For this review, use the dimensioned drawing (mm, ordinates from the lowest corner) and the shaded views. Give positions to 0.01 mm unless a question says otherwise; leave off trailing zeros. Order: outer loops, then holes, each group sorted by start corner. A loop starts at its lowest first (then second) coordinate and runs counter-clockwise, first axis right, second up.
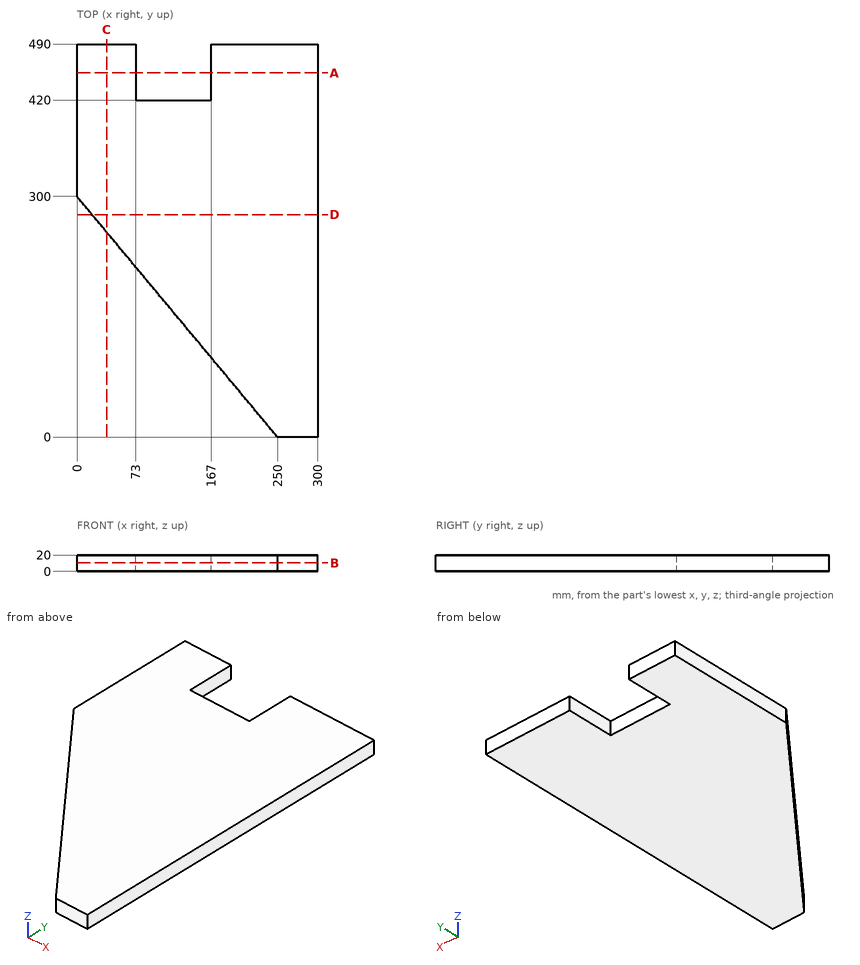
1. Take a section at A-A (y = 454). State the section outline as (x, z) points.
Recorded:
outline: (0, 0) - (73, 0) - (73, 20) - (0, 20) - close; (167, 0) - (300, 0) - (300, 20) - (167, 20) - close
2. Take a section at B-B (z = 10.5). State the section outline as (x, y) points, then the cut area to 3 significant figures.
Recorded:
outline: (0, 300) - (250, 0) - (300, 0) - (300, 490) - (167, 490) - (167, 420) - (73, 420) - (73, 490) - (0, 490) - close
area: 103,000 mm2
3. Take a section at D-D (y = 277.5). State the section outline as (x, z) points.
Recorded:
outline: (18.75, 0) - (300, 0) - (300, 20) - (18.75, 20) - close
4. For pin 1 (5 mm diameter, centred on y = 297, z = 2, fed in from -X), flat-tipped, find the tip position at first contact; note if it passes through.
Recorded:
pin 1: stops at x = 0.42
5. Take a section at C-C (x = 37). State the section outline as (y, z) points.
Recorded:
outline: (255.6, 0) - (490, 0) - (490, 20) - (255.6, 20) - close
6. For line 1 along X through (y, z) = (436.5, 7); line 2 along Y through (x, z) = (102.5, 4.75); line 3 along X through (y, z) = (71.5, 6), list the stretches that pass through material, from the lowest coordinate up.
Recorded:
line 1: x = 0 to 73, 167 to 300
line 2: y = 177 to 420
line 3: x = 190.42 to 300
